Geometry check sheet. Reference: the model listing, model coordinates, mm. Face numbers are marked on the shaded views. Round coordinates to 2 decimals unless told otherwise and drop trailing zeros. Loops run counter-clockwise (first coordinate to the right, second up) from the corner with the lowest first, then second, coordinate; pieces in that order, holes last. Notation, with made-up numbers: (44.5, -12.75) -> (94.5, -12.75) arc R8 cw to (94.5, -1.75) -> close; hole circle Ø9 at (52.5, 68). An arc over 180 degrees is marked (long way). Use a Markdown table: item, result. Add a question column.
Q1. Gauge pin test, flat end, axial feed: P1, Ø2, axis at y = 1.5, z = -4.5, coming from the +X side. Record the tip position at first contact, or that the pin passes through.
Q2. Sectioned sample at B-B, the plane y = -1.1. Enter the section's corners in (x, z).
Q3. Material ranges on L1, parallel to X at y = -1.65, z = 0; L2, parallel to X at y = 1.4, z = 1; L3, parallel to Z at x = -24, y = 0.55, recorded low to high.
Q4. Release check for a two-part mould opening along X. For the marked faces 1, 2, 3 and 4 record: released by +X, released by -X, zero draft, split by the parting line, or undercut.
Q5. Sectioned sample at A-A, the plane z = 0. Enter the section's corners in (x, y).
Q6. Sectioned sample at C-C, the plane x = 27.5. Enter the section's corners in (y, z).
Q7. Sectioned sample at D-D, the plane z = -2.5. Enter the section's corners in (x, y).
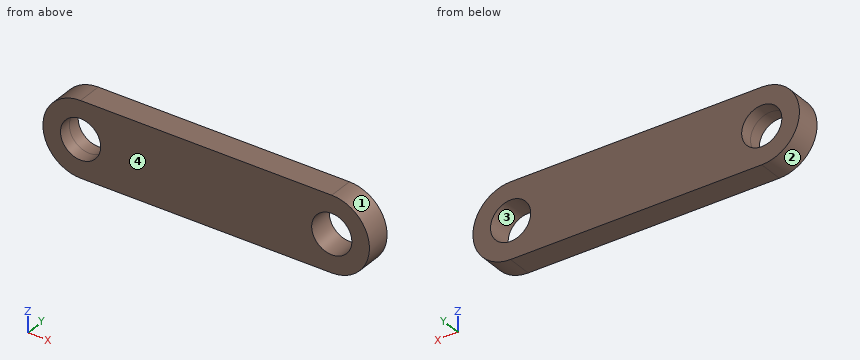
```python
from build123d import *

# Parameters (mm, degrees)
LINK_PLATE_DEPTH     = 2.5
PIN_HOLES_SKETCH_R   = 4
PIN_HOLES_2X_8_DEPTH = 2.5


with BuildPart() as part:
    # Link Profile Sketch → Link Plate (new, symmetric)
    with BuildSketch(Plane(origin=(0, 0, 0), x_dir=(1, 0, 0), z_dir=(0, 1, 0))):
        with BuildLine():
            Line((-25, 7.5), (25, 7.5))
            ThreePointArc((25, 7.5), (32.5, 0), (25, -7.5))
            Line((25, -7.5), (-25, -7.5))
            ThreePointArc((-25, -7.5), (-32.5, 0), (-25, 7.5))
        make_face()
    extrude(amount=LINK_PLATE_DEPTH, both=True)

    # Pin Holes Sketch → Pin Holes 2xØ8 (cut, symmetric)
    with BuildSketch(Plane(origin=(0, 0, 0), x_dir=(1, 0, 0), z_dir=(0, 1, 0))):
        with Locations(Location((-25, 0, 0), (0, 0, 270))):
            Circle(PIN_HOLES_SKETCH_R)
        with Locations(Location((25, 0, 0), (0, 0, 270))):
            Circle(PIN_HOLES_SKETCH_R)
    extrude(amount=PIN_HOLES_2X_8_DEPTH, both=True, mode=Mode.SUBTRACT)


solid = part.part
```
Values:
| question | item | result |
|---|---|---|
| 1 | P1 | x = 31.63 |
| 2 | outline | (-25, -7.5) -> (25, -7.5) arc R7.5 ccw to (25, 7.5) -> (-25, 7.5) arc R7.5 ccw to start; hole circle Ø8 at (-25, 0); hole circle Ø8 at (25, 0) |
| 3 | L1 | -32.5 to -29, -21 to 21, 29 to 32.5 |
| 3 | L2 | -32.43 to -28.87, -21.13 to 21.13, 28.87 to 32.43 |
| 3 | L3 | -7.5 to -3.87, 3.87 to 7.5 |
| 4 | face 1 | released by +X |
| 4 | face 2 | released by -X |
| 4 | face 3 | undercut |
| 4 | face 4 | zero draft |
| 5 | outline | (-32.5, -2.5) -> (-29, -2.5) -> (-29, 2.5) -> (-32.5, 2.5) -> close; (-21, -2.5) -> (21, -2.5) -> (21, 2.5) -> (-21, 2.5) -> close; (29, -2.5) -> (32.5, -2.5) -> (32.5, 2.5) -> (29, 2.5) -> close |
| 6 | outline | (-2.5, -7.07) -> (2.5, -7.07) -> (2.5, -3.12) -> (-2.5, -3.12) -> close; (-2.5, 3.12) -> (2.5, 3.12) -> (2.5, 7.07) -> (-2.5, 7.07) -> close |
| 7 | outline | (-32.07, -2.5) -> (-28.12, -2.5) -> (-28.12, 2.5) -> (-32.07, 2.5) -> close; (-21.88, -2.5) -> (21.88, -2.5) -> (21.88, 2.5) -> (-21.88, 2.5) -> close; (28.12, -2.5) -> (32.07, -2.5) -> (32.07, 2.5) -> (28.12, 2.5) -> close |
